from build123d import *

# Parameters (mm, degrees)
SKETCH_1_W                   = 60
SKETCH_1_H                   = 50
EXTRUDE_1_DEPTH              = 6
SKETCH_2_W                   = 60
SKETCH_2_H                   = 12
CUT_EXTRUDE_1_DEPTH          = 2
CUT_EXTRUDE_2_DEPTH          = 41.853396432
HOLE_WIZARD_M4_1_D           = 5.5
HOLE_WIZARD_M4_1_CBORE_D     = 10
HOLE_WIZARD_M4_1_CBORE_DEPTH = 5.4


with BuildPart() as part:
    # 草图1 → 凸台-拉伸1 (new, symmetric)
    with BuildSketch(Plane.XY):
        Rectangle(SKETCH_1_W, SKETCH_1_H)
    extrude(amount=EXTRUDE_1_DEPTH, both=True)

    # 草图2 → 切除-拉伸1 (cut)
    with BuildSketch(Plane.XY.offset(6)):
        with Locations((0, 19)):
            Rectangle(SKETCH_2_W, SKETCH_2_H)
    extrude(amount=-CUT_EXTRUDE_1_DEPTH, mode=Mode.SUBTRACT)

    # 草图3 → 切除-拉伸2 (cut, through all)
    with BuildSketch(Plane.XY.offset(6)):
        with BuildLine():
            Line((-17.7, -19), (-17.7, 6))
            ThreePointArc((-17.7, 6), (-15, 8.7), (-12.3, 6))
            Line((-12.3, 6), (-12.3, -19))
            ThreePointArc((-12.3, -19), (-15, -21.7), (-17.7, -19))
        make_face()
        with BuildLine():
            Line((12.3, -19), (12.3, 6))
            ThreePointArc((12.3, 6), (15, 8.7), (17.7, 6))
            Line((17.7, 6), (17.7, -19))
            ThreePointArc((17.7, -19), (15, -21.7), (12.3, -19))
        make_face()
    extrude(amount=-CUT_EXTRUDE_2_DEPTH, mode=Mode.SUBTRACT)

    # M4 沉头孔1 (through all)
    with Locations(Plane(origin=(0, 0, -6), x_dir=(-1, 0, 0), z_dir=(0, 0, -1))):
        with Locations((-15, 19), (15, 19)):
            CounterBoreHole(HOLE_WIZARD_M4_1_D / 2, HOLE_WIZARD_M4_1_CBORE_D / 2, HOLE_WIZARD_M4_1_CBORE_DEPTH)


solid = part.part
Design review of the part built by this model. Coordinates are the model's own, in mm. A direction names the side the tool comes from. Give positions to 0.01 mm unless a question says otherwise; leave off trailing zeros. Write each loop counter-clockwise with the first axis right and the second up, starting at its lowest first coordinate (ties: lowest second). Pieces come first, ordered by that corner, then holes. Notation, with made-up numbers: M 68,18 L 113,18 A35 ccw 113,56 Z; hole C 41.25,-35.5 d7. An arc over 180 degrees is marked long. Answer as a JSON object with one key per item and string values. Group by question number.
1) Clearance check with flat-ended pins moving along their axes: pin 1 Ø3.5 at (x, y) = (9.5, 18) entering from +Z; pin 2 Ø4.5 at (x, y) = (-15, 19) entering from -Z; pin 3 Ø8 at (x, y) = (15, 19) entering from -Z. State where each tip first meets the part, or that it passes through.
2) For line 1 along X through (y, z) = (6, 5); line 2 along Y through (x, z) = (-15, 2.8); line 3 along Y through (x, z) = (-16, 0.5), list the stretches that pass through material, from the lowest coordinate up.
3) Tool access review of faces 1 (the face through (-12.3, -6, 0)), 2 (the face through (16.08, 14.12, -3.34)), 3 (the face through (0, 13, 5)), 4 (the face through (0, -6, 6)), 5 (the face through (0, 0, -6)): name each direction out of +Z, -Z, +X, -X, +Y, -Y from which nothing blocks a thin tool from reaching the whole face with its end or side.
4) Mouldability with a two-part tool opening along X and no side actions: class faces 6 (the face through (30, 0, 0)), 7 (the face through (-15.1, 8.7, 0.1)), 8 (the face through (-14.9, -21.7, 0.1)), 9 (the face through (0, 19, 4)) as released by +X, released by -X, zero draft, split by the parting line, or undercut.
5) We need section C-C (z = 0.25). Give the boundary of the cut face in (x, y), and give its area (3 significant figures).
6) We need section B-B (x = 15). Give the boundary of the cut face in (y, z).
7) We need section A-A (y = 19). Give the boundary of the cut face in (x, z), and give its area (3 significant figures).
8) We need section D-D (y = -11.5). Give the boundary of the cut face in (x, z).
Answer key:
{
 "1": {"pin 1": "stops at z = 4", "pin 2": "passes through", "pin 3": "stops at z = -0.6"},
 "2": {"line 1": "x = -30 to -17.7, -12.3 to 12.3, 17.7 to 30", "line 2": "y = -25 to -21.7, 8.7 to 16.25, 21.75 to 25", "line 3": "y = -25 to -21.51, 8.51 to 16.44, 21.56 to 25"},
 "3": {"face 1": "+Z, -Z", "face 2": "-Z", "face 3": "+Z, +X, -X, +Y", "face 4": "+Z, +X, -X, +Y, -Y", "face 5": "-Z, +X, -X, +Y, -Y"},
 "4": {"face 6": "released by +X", "face 7": "undercut", "face 8": "undercut", "face 9": "zero draft"},
 "5": {"outline": "M -30,-25 L 30,-25 L 30,25 L -30,25 Z; hole C -15,19 d5.5; hole M -17.7,-19 A2.7 ccw -12.3,-19 L -12.3,6 A2.7 ccw -17.7,6 Z; hole C 15,19 d5.5; hole M 12.3,-19 A2.7 ccw 17.7,-19 L 17.7,6 A2.7 ccw 12.3,6 Z", "area": "2,640 mm²"},
 "6": {"outline": "M -25,-6 L -21.7,-6 L -21.7,6 L -25,6 Z; M 8.7,-6 L 14,-6 L 14,-0.6 L 16.25,-0.6 L 16.25,4 L 13,4 L 13,6 L 8.7,6 Z; M 21.75,-0.6 L 24,-0.6 L 24,-6 L 25,-6 L 25,4 L 21.75,4 Z"},
 "7": {"outline": "M -30,-6 L -20,-6 L -20,-0.6 L -17.75,-0.6 L -17.75,4 L -30,4 Z; M -12.25,-0.6 L -10,-0.6 L -10,-6 L 10,-6 L 10,-0.6 L 12.25,-0.6 L 12.25,4 L -12.25,4 Z; M 17.75,-0.6 L 20,-0.6 L 20,-6 L 30,-6 L 30,4 L 17.75,4 Z", "area": "441 mm²"},
 "8": {"outline": "M -30,-6 L -17.7,-6 L -17.7,6 L -30,6 Z; M -12.3,-6 L 12.3,-6 L 12.3,6 L -12.3,6 Z; M 17.7,-6 L 30,-6 L 30,6 L 17.7,6 Z"}
}
